```python
from build123d import *

# Parameters (mm, degrees)
EXTRUDE_1_DEPTH              = 17.5
HOLE_WIZARD_M4_1_D           = 3.3
HOLE_WIZARD_M4_1_DEPTH       = 9.5
HOLE_WIZARD_M4_1_TIP         = 0.991420021
HOLE_WIZARD_M6_1_D           = 5
HOLE_WIZARD_M6_1_DEPTH       = 12
HOLE_WIZARD_M6_1_CSINK_D     = 6.05
HOLE_WIZARD_M6_1_CSINK_ANGLE = 90
HOLE_WIZARD_M6_1_TIP         = 1.502151548


with BuildPart() as part:
    # 草图1 → 凸台-拉伸1 (new, symmetric)
    with BuildSketch(Plane.XY):
        with BuildLine():
            Line((-27.5, 27), (27.5, 27))
            Line((27.5, 27), (27.5, -17))
            Line((27.5, -17), (9, -17))
            Line((9, -17), (9, -10.723805295))
            ThreePointArc((9, -10.723805295), (0, 14), (-9, -10.723805295))
            Line((-9, -10.723805295), (-9, -17))
            Line((-9, -17), (-27.5, -17))
            Line((-27.5, -17), (-27.5, 27))
        make_face()
    extrude(amount=EXTRUDE_1_DEPTH, both=True)

    # M4 螺纹孔1
    with Locations(Plane.XY.offset(17.5)):
        with Locations((18.186533479, 10.5), (18.186533479, -10.5), (-18.186533479, -10.5), (-18.186533479, 10.5)):
            Hole(HOLE_WIZARD_M4_1_D / 2, depth=HOLE_WIZARD_M4_1_DEPTH)
            with Locations((0, 0, -(HOLE_WIZARD_M4_1_DEPTH + HOLE_WIZARD_M4_1_TIP / 2))):  # 118° drill point
                Cone(0, HOLE_WIZARD_M4_1_D / 2, HOLE_WIZARD_M4_1_TIP, mode=Mode.SUBTRACT)

    # M6 螺纹孔1
    with Locations(Plane(origin=(-20.5, 27, 10.5), x_dir=(0, 0, 1), z_dir=(0, 1, 0))):
        with Locations((0, 0), (-21, 0), (-21, 41), (0, 41)):
            CounterSinkHole(HOLE_WIZARD_M6_1_D / 2, HOLE_WIZARD_M6_1_CSINK_D / 2, depth=HOLE_WIZARD_M6_1_DEPTH, counter_sink_angle=HOLE_WIZARD_M6_1_CSINK_ANGLE)
            with Locations((0, 0, -(HOLE_WIZARD_M6_1_DEPTH + HOLE_WIZARD_M6_1_TIP / 2))):  # 118° drill point
                Cone(0, HOLE_WIZARD_M6_1_D / 2, HOLE_WIZARD_M6_1_TIP, mode=Mode.SUBTRACT)


solid = part.part
```
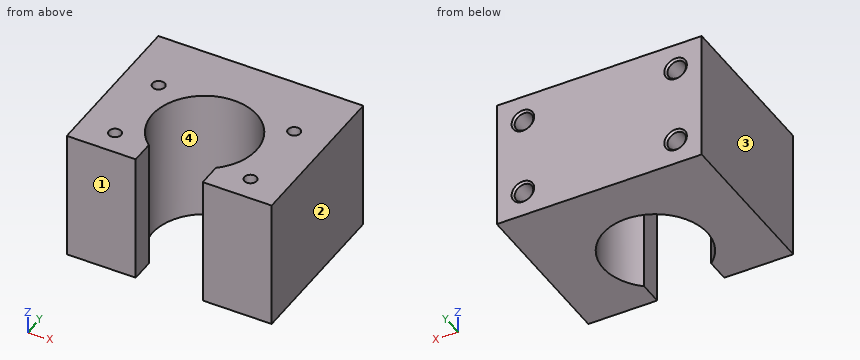
Geometry: final body of the model. Coordinates: model frame, mm. Face numbers are marked on the shaded views. Coordinates: 2 decimals unless noted, no trailing zeros. Order: outer loops, then holes, each group sorted by start corner. A loop starts at its lowest first (then second) coordinate and runs counter-clockwise, first axis right, second up.
Item 1: Section query C-C (y = 24). Output: boundary loops of the cut face in (x, z).
Answer:
outline: (-27.5, -17.5) - (27.5, -17.5) - (27.5, 17.5) - (-27.5, 17.5) - close; hole circle Ø5 at (-20.5, -10.5); hole circle Ø5 at (-20.5, 10.5); hole circle Ø5 at (20.5, -10.5); hole circle Ø5 at (20.5, 10.5)
Item 2: Section query A-A (y = 0). Output: boundary loops of the cut face in (x, z).
Answer:
outline: (-27.5, -17.5) - (-14, -17.5) - (-14, 17.5) - (-27.5, 17.5) - close; (14, -17.5) - (27.5, -17.5) - (27.5, 17.5) - (14, 17.5) - close
Item 3: Draft query along X for the marked faces 1, 2, 3 and 4. Return one class per face: released by +X, released by -X, zero draft, split by the parting line, or undercut.
Answer:
face 1: zero draft
face 2: released by +X
face 3: released by -X
face 4: undercut
Item 4: Contact query for flat-ended pins moving along their axis: P1, Ø3, axis at x = 20.5, z = 10.5, coming from the +Y side; P2, Ø2.5, axis at x = 18.19, y = 10.5, coming from the +Z side. Output: stop coordinate, or through.
Answer:
P1: stops at y = 14.4
P2: stops at z = 7.76
Item 5: Material intervals for line 1 along Z through (x, y) = (20.5, 18.5); line 2 along X through (y, z) = (18.75, -10.5); line 3 along Z through (x, y) = (20, 23), sorted ascending.
Answer:
line 1: z = -17.5 to -13, -8 to 8, 13 to 17.5
line 2: x = -27.5 to -23, -18 to 18, 23 to 27.5
line 3: z = -17.5 to -12.95, -8.05 to 8.05, 12.95 to 17.5
Item 6: Section query D-D (z = -1.5). Output: boundary loops of the cut face in (x, y).
Answer:
outline: (-27.5, -17) - (-9, -17) - (-9, -10.72) arc R14 cw (long way) to (9, -10.72) - (9, -17) - (27.5, -17) - (27.5, 27) - (-27.5, 27) - close
Item 7: Section query B-B (x = -10). Output: boundary loops of the cut face in (y, z).
Answer:
outline: (-17, -17.5) - (-9.8, -17.5) - (-9.8, 17.5) - (-17, 17.5) - close; (9.8, -17.5) - (27, -17.5) - (27, 17.5) - (9.8, 17.5) - close
